Check sheet for the drawn part. Datum: minimum x, y, z corner. Units: mm. A direction names the side the tool comes from. Coordinates: 2 decimals unless noted, no trailing zeros. Write each loop counter-clockwise with the first axis right and the second up, starting at its lowest first coordinate (ties: lowest second). Pieces come first, ordered by that corner, then holes. Notation, with made-up numbers: M 17.25,-37 L 38.25,-37 A21 ccw 38.25,-8 Z; hole C -17,84.5 d11. An arc over 180 degrees is marked long. Answer in a Markdown table with one row per item.
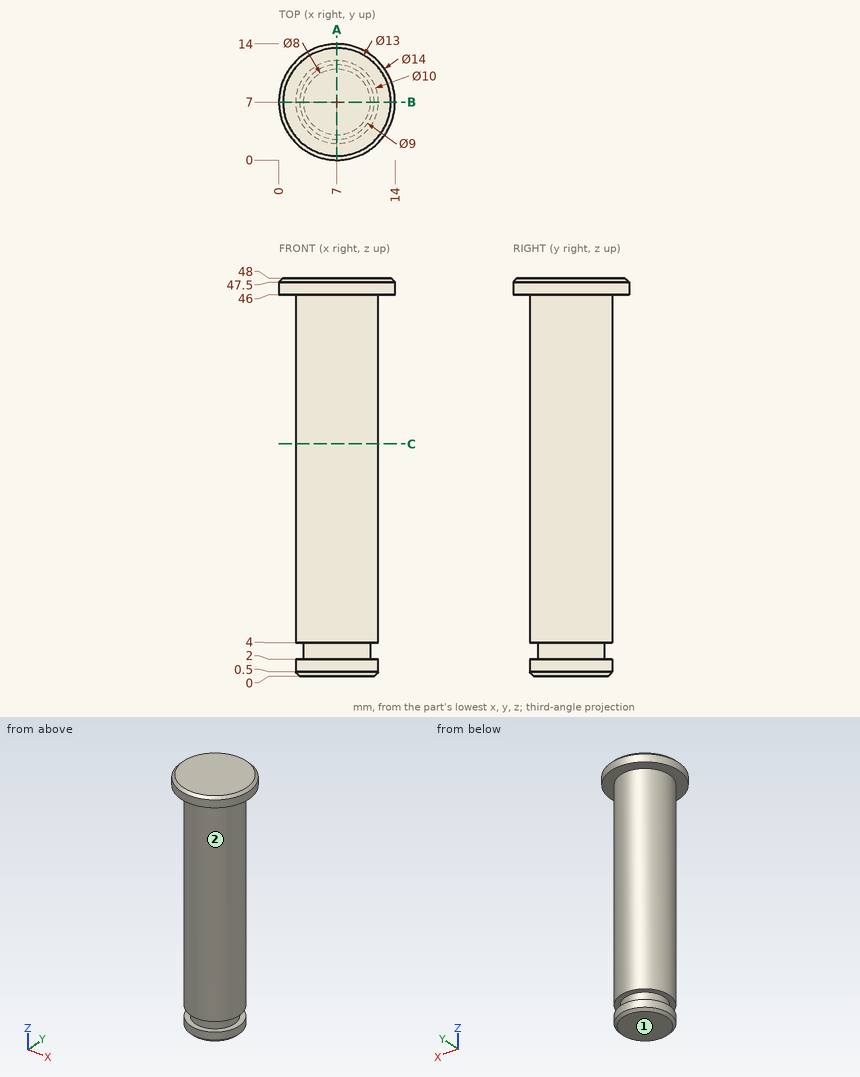
1) Tool access check on the marked faces 1 and 2. Record the directions out of +Z, -Z, +X, -X, +Y, -Y that give a thin tool (end or side, any length) a straight path to the whole face; none if there is none.
Response values:
| item | result |
|---|---|
| face 1 | -Z, +X, -X, +Y, -Y |
| face 2 | -Z |
2) Sectioned sample at A-A (x = 7). Record the cut outline in (y, z).
Response values:
| item | result |
|---|---|
| outline | M 0,46 L 2,46 L 2,4 L 3,4 L 3,2 L 2,2 L 2,0.5 L 2.5,0 L 11.5,0 L 12,0.5 L 12,2 L 11,2 L 11,4 L 12,4 L 12,46 L 14,46 L 14,47.5 L 13.5,48 L 0.5,48 L 0,47.5 Z |
3) Sectioned sample at C-C (z = 28). Record the cut outline in (x, y).
Response values:
| item | result |
|---|---|
| outline | C 7,7 d10 |
4) Depth check by flat-ended pin: pin 1 (1.5 mm diameter, centred on x = 2.5, z = 7.5, fed in from +Y); pin 2 (1.5 mm diameter, centred on x = 3, z = 7.5, fed in from +Y); pin 3 (1 mm diameter, centred on x = 8, z = 34.5, fed in from -Y). Enter the tip coordinate at first touch or a pass-through.
Response values:
| item | result |
|---|---|
| pin 1 | stops at y = 10.31 |
| pin 2 | stops at y = 10.8 |
| pin 3 | stops at y = 2.03 |
5) Thickness scan on L1, parallel to Z at x = 6.25, y = 3; L2, parallel to Z at x = 2.25, y = 4.75; L3, parallel to X at y = 11.5, z = 21. Record the ranges inside material, lowest first. Write a range as [from, to].
Response values:
| item | result |
|---|---|
| L1 | z = [0, 2], [4, 48] |
| L2 | z = [46, 48] |
| L3 | x = [4.82, 9.18] |
